Could you check a few things on this model? Use its own coordinates, in mm. A direction names the side the tool comes from. Give positions to 0.01 mm unless a question says otherwise; leave off trailing zeros. Loops run counter-clockwise (first coordinate to the right, second up) from the corner with the lowest first, then second, coordinate; pieces in that order, holes last. Notation, with made-up numbers: M -26,18 L 25,18 A34 cw 25,55 Z; hole C -31,-31 d5. An arc over 180 degrees is marked long. Use a Markdown table: item, result. Add a question column.
1) Suppose I cut it at D-D on x = 57. List the corners of the cut face in (y, z) for me.
2) Suppose I cut it at B-B on y = 67. List the corners of the cut face in (x, z) for me, and give its area (3 significant figures).
3) We'd pull the mould along X, two halves only. Please class faces 1 (the flat face through (86, 81.5, 5)), 2 (the cylindrical face through (88.503, 40.486, 4.93)), 3 (the cylindrical face through (105.619, 67.585, 5.07)), 4 (the flat face through (47, 76, 5)): +X half, -X half, draft (parallel to the pull), parting line (faces both ways), or undercut.
4) If I drill on line 1 along Y through (x, z) = (101, 6); line 2 along X through (y, z) = (14, 4.75); line 3 along Y through (x, z) = (6.5, 0.5), over which ranges is the centre line in solid material (lowest first)? Write a range as [from, to].
5) Which directions (+Z, -Z, +X, -X, +Y, -Y) give clear straight access to the entire face, cutting with the end or side of a thin tool? Please do faces 5 (the flat face through (47, 5, 5)), 6 (the cylindrical face through (110.99, 2.85, 5.07)), 7 (the flat face through (7, 52.75, 5)), 8 (the cylindrical face through (111.15, 78.49, 5.07)), 9 (the flat face through (67, 77, 5)).
6) Will these pins go through, and if not, where does the flat tip stop? pin 1 Ø3 at (x, z) = (5, 3.5) entering from +Y; pin 2 Ø9 at (x, y) = (13, 12) entering from -Z; pin 3 Ø3 at (x, z) = (108, 4.5) entering from +Y; pin 4 Ø3 at (x, z) = (5, 3.5) entering from -Y.
7) Suppose I cut it at A-A on z = 7. List the corners of the cut face in (x, y) for me, and give its area (3 significant figures).
8) Suppose I cut it at C-C on y = 18.5. List the corners of the cut face in (x, z) for me, and give its area (3 significant figures).
```python
from build123d import *

# Parameters (mm, degrees)
BRACKET_PLATE_DEPTH        = 10
MOUNTING_HOLES_SKETCH_R    = 5
MOUNTING_HOLES_4X_10_DEPTH = 141.492882382
CORNER_FILLETS_R10_R       = 10


with BuildPart() as part:
    # Bracket Profile Sketch → Bracket Plate (new body)
    with BuildSketch(Plane.XY):
        with BuildLine():
            Line((10, 0), (47, 0))
            Line((47, 0), (47, 10))
            ThreePointArc((47, 10), (57, 20), (67, 10))
            Line((67, 10), (67, 0))
            Line((67, 0), (104, 0))
            Line((104, 0), (114, 0))
            Line((114, 0), (114, 10))
            Line((114, 10), (114, 28.75))
            Line((114, 28.75), (100.5, 28.75))
            ThreePointArc((100.5, 28.75), (88.5, 40.75), (100.5, 52.75))
            Line((100.5, 52.75), (114, 52.75))
            Line((114, 52.75), (114, 71.5))
            Line((114, 71.5), (114, 81.5))
            Line((114, 81.5), (104, 81.5))
            Line((104, 81.5), (67, 81.5))
            Line((67, 81.5), (67, 71.5))
            ThreePointArc((67, 71.5), (57, 61.5), (47, 71.5))
            Line((47, 71.5), (47, 81.5))
            Line((47, 81.5), (10, 81.5))
            Line((10, 81.5), (0, 81.5))
            Line((0, 81.5), (0, 71.5))
            Line((0, 71.5), (0, 52.75))
            Line((0, 52.75), (13.5, 52.75))
            ThreePointArc((13.5, 52.75), (25.5, 40.75), (13.5, 28.75))
            Line((13.5, 28.75), (0, 28.75))
            Line((0, 28.75), (0, 10))
            Line((0, 10), (0, 0))
            Line((0, 0), (10, 0))
        make_face()
    extrude(amount=BRACKET_PLATE_DEPTH)

    # Mounting Holes Sketch → Mounting Holes 4xØ10 (cut, through all)
    with BuildSketch(Plane.XY.offset(10)):
        with Locations((13, 69.5)):
            Circle(MOUNTING_HOLES_SKETCH_R)
        with Locations((101, 69.5)):
            Circle(MOUNTING_HOLES_SKETCH_R)
        with Locations((101, 12)):
            Circle(MOUNTING_HOLES_SKETCH_R)
        with Locations((13, 12)):
            Circle(MOUNTING_HOLES_SKETCH_R)
    extrude(amount=-MOUNTING_HOLES_4X_10_DEPTH, mode=Mode.SUBTRACT)

    # Corner Fillets R10
    corner_fillets_r10_edges = [part.edges().sort_by_distance(p)[0] for p in [
        (0, 0, 5),
        (0, 81.5, 5),
        (114, 81.5, 5),
        (114, 0, 5),
    ]]
    fillet(corner_fillets_r10_edges, radius=CORNER_FILLETS_R10_R)


solid = part.part
```
Answer block:
| question | item | result |
|---|---|---|
| 1 | outline | M 20,0 L 61.5,0 L 61.5,10 L 20,10 Z |
| 2 | outline | M 0,0 L 8.67,0 L 8.67,10 L 0,10 Z; M 17.33,0 L 48.07,0 L 48.07,10 L 17.33,10 Z; M 65.93,0 L 96.67,0 L 96.67,10 L 65.93,10 Z; M 105.33,0 L 114,0 L 114,10 L 105.33,10 Z |
| 2 | area | 788 mm^2 |
| 3 | face 1 | draft |
| 3 | face 2 | +X half |
| 3 | face 3 | undercut |
| 3 | face 4 | undercut |
| 4 | line 1 | y = [0, 7], [17, 28.75], [52.75, 64.5], [74.5, 81.5] |
| 4 | line 2 | x = [0, 8.42], [17.58, 47.83], [66.17, 96.42], [105.58, 114] |
| 4 | line 3 | y = [0.63, 28.75], [52.75, 80.87] |
| 5 | face 5 | +Z, -Z, -Y |
| 5 | face 6 | +Z, -Z, +X, -Y |
| 5 | face 7 | +Z, -Z, -X |
| 5 | face 8 | +Z, -Z, +X, +Y |
| 5 | face 9 | +Z, -Z, +Y |
| 6 | pin 1 | stops at y = 80.87 |
| 6 | pin 2 | passes through |
| 6 | pin 3 | stops at y = 81.18 |
| 6 | pin 4 | stops at y = 0.63 |
| 7 | outline | M 0,10 A10 ccw 10,0 L 47,0 L 47,10 A10 cw 67,10 L 67,0 L 104,0 A10 ccw 114,10 L 114,28.75 L 100.5,28.75 A12 cw 100.5,52.75 L 114,52.75 L 114,71.5 A10 ccw 104,81.5 L 67,81.5 L 67,71.5 A10 cw 47,71.5 L 47,81.5 L 10,81.5 A10 ccw 0,71.5 L 0,52.75 L 13.5,52.75 A12 cw 13.5,28.75 L 0,28.75 Z; hole C 13,12 d10; hole C 13,69.5 d10; hole C 101,12 d10; hole C 101,69.5 d10 |
| 7 | area | 7,080 mm^2 |
| 8 | outline | M 0,0 L 51.73,0 L 51.73,10 L 0,10 Z; M 62.27,0 L 114,0 L 114,10 L 62.27,10 Z |
| 8 | area | 1,030 mm^2 |
